Work out the finished part from the listing and answer in its coordinate system (mm). Round coordinates to 2 decimals unless told otherwise and drop trailing zeros. Order: outer loops, then holes, each group sorted by start corner. A loop starts at its lowest first (then second) coordinate and runs counter-clockwise, first axis right, second up. Notation, with made-up numbers: (38.5, 62) - (88.5, 62) arc R23 ccw to (88.5, 91) - close; hole circle Ø1 at (4, -27). An arc over 180 degrees is marked (long way). One line per question, with ' | ' between items. Start each with the question number.
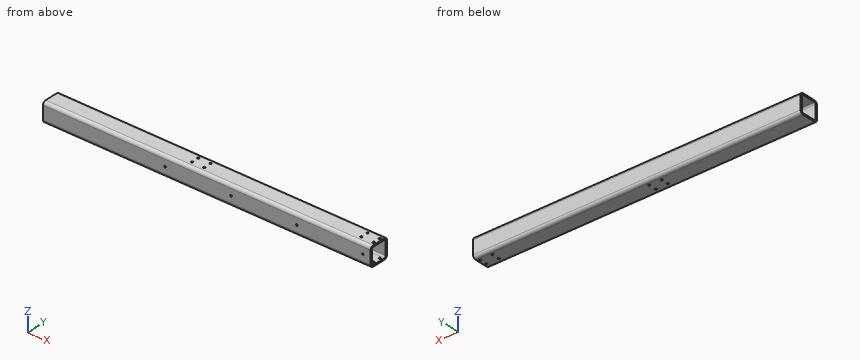
from build123d import *

# Parameters (mm, degrees)
GB_6728_1986_050_X_50_X_4_1_DEPTH = 845
HOLE_WIZARD_M6_1_D                = 5
HOLE_WIZARD_M5_1_D                = 4.2
HOLE_WIZARD_M5_1_DEPTH            = 4


with BuildPart() as part:
    # Sketch1 → Gb／6728-1986方形空心型钢 050 X 50 X 4(1) (new body)
    with BuildSketch(Plane.ZY):
        with BuildLine():
            Line((-17, -25), (17, -25))
            ThreePointArc((17, -25), (22.656854249, -22.656854249), (25, -17))
            Line((25, -17), (25, 17))
            ThreePointArc((25, 17), (22.656854249, 22.656854249), (17, 25))
            Line((17, 25), (-17, 25))
            ThreePointArc((-17, 25), (-22.656854249, 22.656854249), (-25, 17))
            Line((-25, 17), (-25, -17))
            ThreePointArc((-25, -17), (-22.656854249, -22.656854249), (-17, -25))
        make_face()
        with BuildLine():
            Line((-17, -21), (17, -21))
            ThreePointArc((17, -21), (19.828427125, -19.828427125), (21, -17))
            Line((21, -17), (21, 17))
            ThreePointArc((21, 17), (19.828427125, 19.828427125), (17, 21))
            Line((17, 21), (-17, 21))
            ThreePointArc((-17, 21), (-19.828427125, 19.828427125), (-21, 17))
            Line((-21, 17), (-21, -17))
            ThreePointArc((-21, -17), (-19.828427125, -19.828427125), (-17, -21))
        make_face(mode=Mode.SUBTRACT)
    extrude(amount=GB_6728_1986_050_X_50_X_4_1_DEPTH)

    # M6 螺纹孔1 (through all)
    with Locations(Plane(origin=(0, 0, -25), x_dir=(-1, 0, 0), z_dir=(0, 0, -1))):
        with Locations((6.4, 10.6), (6.4, -8.4), (38, 10.6), (38, -8.4), (443, 10.6), (443, -8.4), (474.6, 10.6), (474.6, -8.4)):
            Hole(HOLE_WIZARD_M6_1_D / 2)

    # M5 螺纹孔1
    with Locations(Plane(origin=(0, -25, 0), x_dir=(-1, 0, 0), z_dir=(0, -1, 0))):
        with Locations((20, 0), (190, 0), (360, 0), (530, 0)):
            Hole(HOLE_WIZARD_M5_1_D / 2, depth=HOLE_WIZARD_M5_1_DEPTH)


solid = part.part
1) Flat-ended cylindrical pins translate along their axes: pin 1 (3 mm diameter, centred on x = -474.6, y = -8.4, fed in from +Z); pin 2 (2 mm diameter, centred on x = -413, z = 20, fed in from +Y). Find the tip coordinate at first contact, or state that the pin passes through.
2) Section A-A on x = -759.5 is taken. Give the vertices of the cut face in (y, z), and give its area (3 significant figures).
3) Straight lines are drawn through the part: line 1 (Y direction, x = -6.4, z = 23.95); line 2 (X direction, y = 10, z = 22); line 3 (Y direction, x = -38, z = 22.85). For each, find the intervals that lie inside material, in ascending order.
Recorded:
1) pin 1: passes through | pin 2: stops at y = 24.75
2) outline: (-25, -17) arc R8 ccw to (-17, -25) - (17, -25) arc R8 ccw to (25, -17) - (25, 17) arc R8 ccw to (17, 25) - (-17, 25) arc R8 ccw to (-25, 17) - close; hole (-21, -17) arc R4 ccw to (-17, -21) - (17, -21) arc R4 ccw to (21, -17) - (21, 17) arc R4 ccw to (17, 21) - (-17, 21) arc R4 ccw to (-21, 17) - close | area: 695 mm²
3) line 1: y = -20.96 to -10.9, -5.9 to 8.1, 13.1 to 20.96 | line 2: x = -845 to -477.03, -472.17 to -445.43, -440.57 to -40.43, -35.57 to -8.83, -3.97 to 0 | line 3: y = -22.46 to -10.9, -5.9 to 8.1, 13.1 to 22.46
